Read the model definition and answer for the solid it produces. Units are mm, in the model's axes. A direction names the side the tool comes from. Give positions to 0.01 mm unless a question says otherwise; leave off trailing zeros. Write each loop counter-clockwise with the first axis right and the second up, starting at its lowest first coordinate (ties: lowest second). Pieces come first, ordered by that corner, then holes. Notation, with made-up numbers: (82.25, 56) -> (111.25, 56) arc R26 cw to (111.25, 76) -> close; hole circle Ø11 at (39.5, -37.75). An arc over 180 degrees is marked (long way). Write item = value, one per line.
from build123d import *

# Parameters (mm, degrees)
CUT_EXTRUDE1_DEPTH      = 562.064167453
CUT_EXTRUDE1_DEPTH_BACK = 562.064167453
SKETCH2_W               = 4
SKETCH2_H               = 29
CUT_EXTRUDE2_DEPTH      = 562.064167453
CUT_EXTRUDE2_DEPTH_BACK = 562.064167453
SKETCH3_W               = 4
SKETCH3_H               = 29
CHAMFER1_SIZE           = 3
SKETCH4_R               = 3
CUT_EXTRUDE3_DEPTH      = 4


with BuildPart() as part:
    # Sketch1 → Revolve1 (revolve)
    with BuildSketch(Plane.XY):
        Polygon((0, 561), (4, 561), (4, 537), (6, 522), (6, 0), (0, 0), align=None)
    revolve(axis=Axis((0, -719.526877718, 0), (0, 1, 0)))

    # Sketch2 → Cut-Extrude1 (cut, two sides: drawn at the far end of the back side and taken through both)
    with BuildSketch(Plane.XY.offset(-CUT_EXTRUDE1_DEPTH_BACK)):
        with Locations((-4, 14.5)):
            Rectangle(SKETCH2_W, SKETCH2_H)
    extrude(amount=CUT_EXTRUDE1_DEPTH + CUT_EXTRUDE1_DEPTH_BACK, mode=Mode.SUBTRACT)

    # Sketch3 → Cut-Extrude2 (cut, two sides: drawn at the far end of the back side and taken through both)
    with BuildSketch(Plane.XY.offset(-CUT_EXTRUDE2_DEPTH_BACK)):
        with Locations((4, 14.5)):
            Rectangle(SKETCH3_W, SKETCH3_H)
    extrude(amount=CUT_EXTRUDE2_DEPTH + CUT_EXTRUDE2_DEPTH_BACK, mode=Mode.SUBTRACT)

    # Chamfer1
    chamfer1_edges = [part.edges().sort_by_distance(p)[0] for p in [
        (0, 0, -6),
        (0, 0, 6),
    ]]
    chamfer(chamfer1_edges, length=CHAMFER1_SIZE)

    # Sketch4 → Cut-Extrude3 (cut)
    with BuildSketch(Plane.ZY.offset(2)):
        with Locations((0, 6)):
            Circle(SKETCH4_R)
    extrude(amount=-CUT_EXTRUDE3_DEPTH, mode=Mode.SUBTRACT)


solid = part.part
(1) The part is cut by section B-B on y = 484.5. Determine the outline of the cut face in (x, z).
Checks:
outline = circle Ø12 at (0, 0)
(2) Given P1, Ø1.5, axis at x = 4, z = 2, coming from the -Y side; P2, Ø4, axis at x = 4, y = 418.5, coming from the -Z side; P3, Ø1.5, axis at y = 426, z = 5, coming from the -X side, each flat-ended and moving along its own axis, determine where each tip first touches the part or whether it passes through.
Checks:
P1 = 29
P2 = -5.66
P3 = -4.24
(3) A tool of negligible diameter and unlimited length cuts with its end or side. For faces 1 (the flat face through (2, 14, 0)), 2 (the flat face through (-2, 14, 0)), 3 (the cylindrical face through (-6, 259, 0)), from which of +Z, -Z, +X, -X, +Y, -Y can it reach the whole face along a straight path? Write none if from no direction.
Checks:
face_1 = +Z, -Z, +X, -Y
face_2 = +Z, -Z, -X, -Y
face_3 = +Y, -Y
(4) Consider L1, parallel to Y at x = 0.45, z = 0; L2, parallel to X at y = 233, z = -0.5; L3, parallel to Y at x = 0.75, z = -1.5. Determine where each line is inside the solid, lowest interval first.
Checks:
L1 = 0 to 3, 9 to 561
L2 = -5.98 to 5.98
L3 = 0 to 3.4, 8.6 to 561
(5) The part is cut by section A-A on z = 0. Determine the outline of the cut face in (x, y).
Checks:
outline = (-6, 29) -> (-2, 29) -> (-2, 9) -> (2, 9) -> (2, 29) -> (6, 29) -> (6, 522) -> (4, 537) -> (4, 561) -> (-4, 561) -> (-4, 537) -> (-6, 522) -> close; (-2, 0) -> (2, 0) -> (2, 3) -> (-2, 3) -> close
